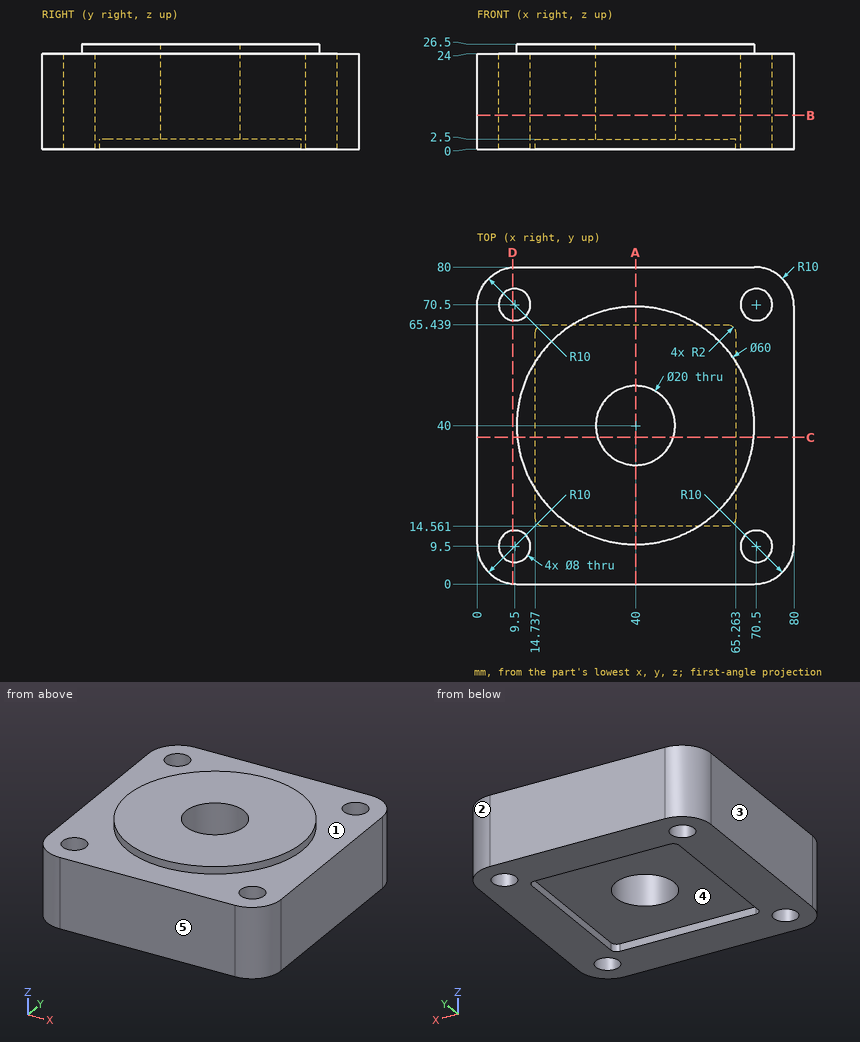
Here's the drawing with two shaded views (mm, measured from the low corner). I have some questions. A direction names the side the tool comes from. Give positions to 0.01 mm unless a question says otherwise; leave off trailing zeros. Order: outer loops, then holes, each group sorted by start corner. A loop starts at its lowest first (then second) coordinate and runs counter-clockwise, first axis right, second up.
Q1. Suppose I cut it at D-D, the plane x = 9. Write out the boundary of the cut face in (y, z).
Q2. I'm going to push flat-ended pins straight in: P1, Ø1.5, axis at x = 70.5, y = 47.5, coming from the +Z side; P2, Ø15, axis at x = 33, y = 33.5, coming from the -Z side. Where does each tip first touch, or does it pass through?
Q3. Suppose I cut it at C-C, the plane y = 37. Write out the boundary of the cut face in (x, z), and give its area (4 significant figures).
Q4. If I drill on line 1 along Y through (x, z) = (70.5, 5.5); line 2 along Y through (x, z) = (40, 17.25); line 3 along X through (y, z) = (73, 19.75) (1 decimal), over which ranges is the centre line in solid material (lowest first)?
Q5. Suppose I cut it at B-B, the plane z = 8.5. Write out the boundary of the cut face in (x, y).
Q6. We'd pull the mould along X, two halves only. Please class the marked faces 3, 4 and 5: +X half, -X half, draft (parallel to the pull), parting line (faces both ways), or undercut.
Q7. Suppose I cut it at A-A, the plane x = 40. Write out the boundary of the cut face in (y, z).
Q8. For the marked faces 1 and 2, which set-ups out of +Z, -Z, +X, -X, +Y, -Y let a thin tool reach every point of the face, with its end or its side?
Solution:
1. outline: (0.05, 0) - (5.53, 0) - (5.53, 24) - (0.05, 24) - close; (13.47, 0) - (66.53, 0) - (66.53, 24) - (13.47, 24) - close; (74.47, 0) - (79.95, 0) - (79.95, 24) - (74.47, 24) - close
2. P1: stops at z = 24
2. P2: stops at z = 2.5
3. outline: (0, 0) - (14.74, 0) - (14.74, 2.5) - (30.46, 2.5) - (30.46, 26.5) - (10.15, 26.5) - (10.15, 24) - (0, 24) - close; (49.54, 2.5) - (65.26, 2.5) - (65.26, 0) - (80, 0) - (80, 24) - (69.85, 24) - (69.85, 26.5) - (49.54, 26.5) - close
3. area: 1,485 mm2
4. line 1: y = 0.01 to 5.5, 13.5 to 66.5, 74.5 to 79.99
4. line 2: y = 0 to 30, 50 to 80
4. line 3: x = 0.5 to 6.4, 12.6 to 67.4, 73.6 to 79.5
5. outline: (0, 10) arc R10 ccw to (10, 0) - (70, 0) arc R10 ccw to (80, 10) - (80, 70) arc R10 ccw to (70, 80) - (10, 80) arc R10 ccw to (0, 70) - close; hole circle Ø8 at (9.5, 9.5); hole circle Ø8 at (9.5, 70.5); hole circle Ø20 at (40, 40); hole circle Ø8 at (70.5, 9.5); hole circle Ø8 at (70.5, 70.5)
6. face 3: -X half
6. face 4: undercut
6. face 5: draft
7. outline: (0, 0) - (14.56, 0) - (14.56, 2.5) - (30, 2.5) - (30, 26.5) - (10, 26.5) - (10, 24) - (0, 24) - close; (50, 2.5) - (65.44, 2.5) - (65.44, 0) - (80, 0) - (80, 24) - (70, 24) - (70, 26.5) - (50, 26.5) - close
8. face 1: +Z
8. face 2: +Z, -Z, +X, +Y
